from build123d import *

# Parameters (mm, degrees)
SKETCH_2_R          = 45
CUT_EXTRUDE_1_DEPTH = 30
CHAMFER_1_SIZE      = 10
CUT_EXTRUDE_2_DEPTH = 2
CHAMFER_2_SIZE      = 2
SKETCH_4_R          = 15
CUT_EXTRUDE_3_DEPTH = 50


with BuildPart() as part:
    # 草图1 → 旋转1 (revolve)
    with BuildSketch(Plane.XY):
        Polygon((0, 0), (0, 175), (20, 175), (20, 110), (48.008301528, 70), (68.008301528, 70), (68.008301528, 50), (88.008301528, 50), (88.008301528, 42.5), (148, 42.5), (148, 40.5), (150, 40.5), (150, 42.5), (200, 42.5), (200, 37.5), (400, 37.5), (400, 0), align=None)
    revolve(axis=Axis((400, 0, 0), (-1, 0, 0)))

    # 草图2 → 切除-拉伸1 (cut)
    with BuildSketch(Plane.ZY):
        with Locations(Location((0, 0, 0), (0, 0, 270))):
            Circle(SKETCH_2_R)
    extrude(amount=-CUT_EXTRUDE_1_DEPTH, mode=Mode.SUBTRACT)

    # 倒角1
    chamfer_1_edges = [part.edges().sort_by_distance(p)[0] for p in [
        (0, 45, 0),
    ]]
    chamfer(chamfer_1_edges, length=CHAMFER_1_SIZE)

    # 草图3 → 切除-拉伸2 (cut)
    with BuildSketch(Plane(origin=(0, 37.5, 0), x_dir=(1, 0, 0), z_dir=(0, 1, 0))):
        with BuildLine():
            Line((333, 10), (385, 10))
            ThreePointArc((385, 10), (395, 0), (385, -10))
            Line((385, -10), (333, -10))
            ThreePointArc((333, -10), (323, 0), (333, 10))
        make_face()
    extrude(amount=-CUT_EXTRUDE_2_DEPTH, mode=Mode.SUBTRACT)

    # 倒角2
    chamfer_2_edges = [part.edges().sort_by_distance(p)[0] for p in [
        (400, -37.5, 0),
    ]]
    chamfer(chamfer_2_edges, length=CHAMFER_2_SIZE)

    # 草图4 → 切除-拉伸3 (cut)
    with BuildSketch(Plane.ZY):
        with Locations(Location((0, 135, 0), (0, 0, 270))):
            Circle(SKETCH_4_R)
        with Locations(Location((95.45941546, 95.45941546, 0), (0, 0, 270))):
            Circle(SKETCH_4_R)
        with Locations(Location((135, 0, 0), (0, 0, 270))):
            Circle(SKETCH_4_R)
        with Locations(Location((95.45941546, -95.45941546, 0), (0, 0, 270))):
            Circle(SKETCH_4_R)
        with Locations(Location((0, -135, 0), (0, 0, 270))):
            Circle(SKETCH_4_R)
        with Locations(Location((-95.45941546, -95.45941546, 0), (0, 0, 270))):
            Circle(SKETCH_4_R)
        with Locations(Location((-135, 0, 0), (0, 0, 270))):
            Circle(SKETCH_4_R)
        with Locations(Location((-95.45941546, 95.45941546, 0), (0, 0, 270))):
            Circle(SKETCH_4_R)
    extrude(amount=-CUT_EXTRUDE_3_DEPTH, mode=Mode.SUBTRACT)


solid = part.part
Read the model definition and answer for the solid it produces. Units are mm, in the model's axes. A direction names the side the tool comes from. Round coordinates to 2 decimals unless told otherwise and drop trailing zeros. Write each loop counter-clockwise with the first axis right and the second up, starting at its lowest first coordinate (ties: lowest second). Pieces come first, ordered by that corner, then holes.
1. Given pin 1 Ø8 at (x, z) = (85.5, -18.5) entering from +Y; pin 2 Ø10 at (x, z) = (168, 16) entering from -Y; pin 3 Ø10 at (x, z) = (372.5, -3.5) entering from +Y; pin 4 Ø24 at (y, z) = (0, -135) entering from -X, each flat-ended and moving along its own axis, determine where each tip first touches the part or whether it passes through.
2. The part is cut by section A-A, the plane y = 0. State how many separate pieces and enclosed holes the cut face has, then the cut area to 3 significant figures.
3. The part is cut by section B-B, the plane y = -126.5. Determine the outline of the cut face in (x, z).
4. Which of the six approach directions +Z, -Z, +X, -X, +Y, -Y give full straight-line access (tool end or side, diameter ignored) to faces 5 (the face through (30, 1, 1)), 6 (the face through (150, -38, 16)), 7 (the face through (118.424, -33.727, 25.861))?
5. Determine the mould class of faces 1 (the face through (360, 35.5, 0)), 2 (the face through (9.86, 1.953, -120.128)), 3 (the face through (149.01, 21.77, -34.15)), 4 (the face through (148, 38, 16)) for opening direction Y: pulls with the +Y half, pulls with the -Y half, needs draft (parallel to the pull), parting line crosses it, or undercut.
6. Straight lines are drawn through the part: L1, parallel to Z at x = 23.75, y = 0; L2, parallel to X at y = -10, z = 18.5; L3, parallel to X at y = 12, z = 148. For each, find the intervals that lie inside material, in ascending order.
7. The part is cut by section C-C, the plane x = 308. Determine the outline of the cut face in (y, z), then the cut area to 3 significant figures.
Values:
1. pin 1: stops at y = 47.85
1. pin 2: stops at y = -41.05
1. pin 3: stops at y = 35.5
1. pin 4: passes through
2. separate pieces: 3
2. enclosed holes: 0
2. area: 37,300 mm2
3. outline: (0, -120.92) - (20, -120.92) - (20, -12.36) - (0, -12.36) - close; (0, 12.36) - (20, 12.36) - (20, 120.92) - (0, 120.92) - close
4. face 5: -X
4. face 6: none
4. face 7: +X
5. face 1: pulls with the +Y half
5. face 2: undercut
5. face 3: parting line crosses it
5. face 4: needs draft
6. L1: z = -104.64 to -45, 45 to 104.64
6. L2: x = 30 to 400
6. L3: x = 0 to 20
7. outline: circle Ø75 at (0, 0)
7. area: 4,420 mm2
